Geometry check sheet. Reference: the model listing, model coordinates, mm. A direction names the side the tool comes from. Coordinates: 2 decimals unless noted, no trailing zeros. Loops run counter-clockwise (first coordinate to the right, second up) from the corner with the lowest first, then second, coordinate; pieces in that order, holes last.
from build123d import *

# Parameters (mm, degrees)
BOSS_EXTRUDE1_DEPTH = 10
SHELL1_T            = -3


with BuildPart() as part:
    # Sketch2 → Boss-Extrude1 (new body)
    with BuildSketch(Plane.XY):
        with BuildLine():
            Line((0, 24), (-260, 24))
            ThreePointArc((-260, 24), (-284, 0), (-260, -24))
            Line((-260, -24), (0, -24))
            ThreePointArc((0, -24), (24, 0), (0, 24))
        make_face()
    extrude(amount=BOSS_EXTRUDE1_DEPTH)

    # Shell1
    shell1_openings = [part.faces().sort_by_distance(p)[0] for p in [
        (-130, 0, 10),
        (-130, 0, 0),
    ]]
    offset(amount=SHELL1_T, openings=shell1_openings, kind=Kind.INTERSECTION)


solid = part.part
(1) Sectioned sample at B-B on z = 8. Record the cut outline in (x, y), and give its area (3 significant figures).
Findings:
outline: (-260, -24) - (0, -24) arc R24 ccw to (0, 24) - (-260, 24) arc R24 ccw to start; hole (-260, -21) - (0, -21) arc R21 ccw to (0, 21) - (-260, 21) arc R21 ccw to start
area: 1,980 mm2
(2) Scan lines: L1, parallel to Y at x = -226, z = 3.5; L2, parallel to X at y = 1, z = 2.75; L3, parallel to X at y = 1.5, z = 7. Record each from-to range of solid material in increasing order.
Findings:
L1: y = -24 to -21, 21 to 24
L2: x = -283.98 to -280.98, 20.98 to 23.98
L3: x = -283.95 to -280.95, 20.95 to 23.95
(3) Gauge pin test, flat end, axial feed: pin 1 Ø2 at (y, z) = (-14.5, 6.5) entering from -X. Record the tip position at first contact, or that the pin passes through.
Findings:
pin 1: stops at x = -279.84
(4) Sectioned sample at C-C on y = 0. Record the cut outline in (x, z).
Findings:
outline: (-284, 0) - (-281, 0) - (-281, 10) - (-284, 10) - close; (21, 0) - (24, 0) - (24, 10) - (21, 10) - close
(5) Draft check along Y on faces 3 (the flat face through (-128, 24, 5)), 4 (the cylindrical face through (-281, 0, 5)), 5 (the cylindrical face through (-283.994, 0.528, 4.93)). Enter one of: +Y half, -Y half, draft (parallel to the pull), parting line (faces both ways), or undercut.
Findings:
face 3: +Y half
face 4: undercut
face 5: parting line
(6) Access from +Z, -Z, +X, -X, +Y, -Y to the whole of each face (thin tool, end or side, straight path). Record for faces 1 (the flat face through (-130.7, 21.4, 0)), 2 (the flat face through (-132, -21, 5)).
Findings:
face 1: -Z, +X, -X, +Y, -Y
face 2: +Z, -Z
(7) Sectioned sample at A-A on x = -80.5. Record the cut outline in (y, z).
Findings:
outline: (-24, 0) - (-21, 0) - (-21, 10) - (-24, 10) - close; (21, 0) - (24, 0) - (24, 10) - (21, 10) - close
